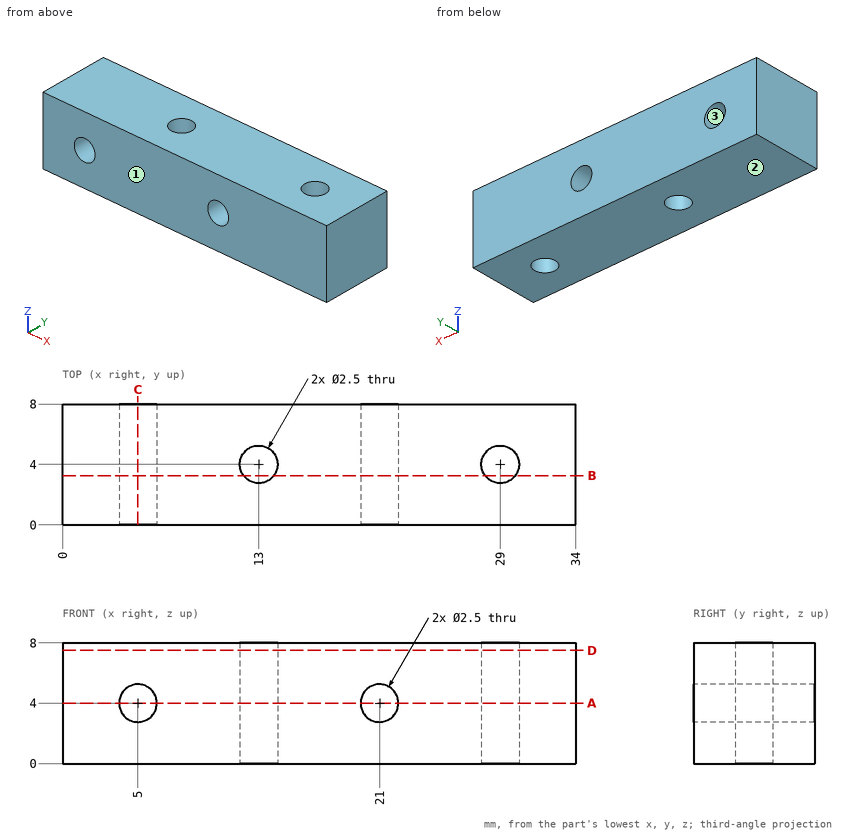
Can you work these out from the drawing? Everything is in mm from the part's minimum corner. Give positions to 0.01 mm unless a question says otherwise; leave off trailing zeros. Order: outer loops, then holes, each group sorted by start corner. A loop starts at its lowest first (then second) coordinate and runs counter-clockwise, first axis right, second up. Notation, with made-up numbers: (52.25, -6.5) -> (66.25, -6.5) arc R25 cw to (66.25, 10.5) -> close; hole circle Ø7 at (-20, 27). An arc over 180 degrees is marked (long way). Return JSON: item names as keys, results as strings.
1. Imagine slicing it at D-D on z = 7.5. List the corners of the cut face in (x, y) for me, then the cut area to 3 significant figures.
Answer list:
{"outline": "(0, 0) -> (34, 0) -> (34, 8) -> (0, 8) -> close; hole circle Ø2.5 at (13, 4); hole circle Ø2.5 at (29, 4)", "area": "262 mm2"}
2. Imagine slicing it at A-A on z = 4. List the corners of the cut face in (x, y) for me, then the cut area to 3 significant figures.
Answer list:
{"outline": "(0, 0) -> (3.75, 0) -> (3.75, 8) -> (0, 8) -> close; (6.25, 0) -> (19.75, 0) -> (19.75, 8) -> (6.25, 8) -> close; (22.25, 0) -> (34, 0) -> (34, 8) -> (22.25, 8) -> close; hole circle Ø2.5 at (13, 4); hole circle Ø2.5 at (29, 4)", "area": "222 mm2"}
3. I need wall thicknesses on line 1 (Z direction, x = 5, y = 6.25); line 2 (X direction, y = 1.25, z = 3.75); line 3 (X direction, y = 5, z = 5.75). Which ranges of each line are inside material? Lowest first, please. Write a range as from..to.
Answer list:
{"line 1": "z = 0..2.75, 5.25..8", "line 2": "x = 0..3.78, 6.22..19.78, 22.22..34", "line 3": "x = 0..12.25, 13.75..28.25, 29.75..34"}
4. Thinking about a two-plate mould opening in Z: for the marked faces 1, 2 and 3, which applies, pulls with the +Z half, pulls with the -Z half, needs draft (parallel to the pull), parting line crosses it, or undercut?
Answer list:
{"face 1": "needs draft", "face 2": "pulls with the -Z half", "face 3": "undercut"}
5. Imagine slicing it at B-B on y = 3.25. List the corners of the cut face in (x, z) for me.
Answer list:
{"outline": "(0, 0) -> (12, 0) -> (12, 8) -> (0, 8) -> close; (14, 0) -> (28, 0) -> (28, 8) -> (14, 8) -> close; (30, 0) -> (34, 0) -> (34, 8) -> (30, 8) -> close; hole circle Ø2.5 at (5, 4); hole circle Ø2.5 at (21, 4)"}
6. Imagine slicing it at C-C on x = 5. List the corners of the cut face in (y, z) for me, then the cut area to 3 significant figures.
Answer list:
{"outline": "(0, 0) -> (8, 0) -> (8, 2.75) -> (0, 2.75) -> close; (0, 5.25) -> (8, 5.25) -> (8, 8) -> (0, 8) -> close", "area": "44.0 mm2"}
7. For pin 1 Ø3 at (x, y) = (13, 4) entering from -Z, with a flat end and sliding along its axis, tell me the tip position at first contact or that it passes through.
Answer list:
{"pin 1": "stops at z = 0"}
